Could you check a few things on this model? Use its own coordinates, in mm. Face numbers are marked on the shaded views. A direction names the side the tool comes from. Round coordinates to 2 decimals unless told otherwise and drop trailing zeros. Loops run counter-clockwise (first coordinate to the right, second up) from the corner with the lowest first, then second, coordinate; pieces in that order, holes last. Notation, with made-up numbers: M 13,89 L 54,89 A18 ccw 54,109 Z; hole C 13,19 d5. An arc over 180 degrees is marked long. One line per item, written item: value. Start each with the question number.
Q1. Which directions (+Z, -Z, +X, -X, +Y, -Y) give clear straight access to the entire face, cutting with the end or side of a thin tool? Please do the marked faces 1 and 2.
Q2. Imagine slicing it at A-A (x = 58). Please give me the cut outline in (y, z).
Q3. I'm going to push flat-ended pins straight in: pin 1 Ø2 at (x, y) = (12, 0) entering from -Z; pin 2 Ø2 at (x, z) = (36.5, -3.5) entering from -Y; pin 3 Ø1 at (y, z) = (5, 3.5) entering from -X; pin 4 Ø8 at (x, y) = (38.5, -3) entering from +Z. Where does each tip first touch, or does it pass through?
Q4. Please list where these lines run through material, in increasing order: line 1 along Y through (x, z) = (17.5, -0.25); line 2 along X through (y, z) = (8, 3.5); line 3 along Z through (x, y) = (38.5, -4.5).
from build123d import *

# Parameters (mm, degrees)
BOSS_EXTRUDE_DEPTH = 7.5
CHAMFER_2_SIZE     = 1.4


with BuildPart() as part:
    # Sketch1 → Boss-Extrude (new body)
    with BuildSketch(Plane(origin=(0, 0, 0), x_dir=(0, 0, -1), z_dir=(1, 0, 0))):
        Polygon((9, 5.196152423), (9, -5.196152423), (0, -10.392304845), (-9, -5.196152423), (-9, 5.196152423), (0, 10.392304845), align=None)
    extrude(amount=BOSS_EXTRUDE_DEPTH)

    # Sketch2 → Boss-Revolve1 (revolve)
    with BuildSketch(Plane.XY, mode=Mode.PRIVATE) as boss_revolve1_sk:
        Polygon((0, 0), (62.5, 0), (62.5, 4.4845), (62.5, 6), (7.5, 6), (0, 6), align=None)
    revolve(boss_revolve1_sk.sketch.rotate(Axis((0, 0, 0), (-1, 0, 0)), 90), axis=Axis((0, 0, 0), (-1, 0, 0)))

    # Sketch3 → Cut-Revolve1 (revolve, cut)
    with BuildSketch(Plane.XY):
        Polygon((0, 9), (3.690598923, 15.392304845), (3.690598923, 20.392304845), (-10, 20.392304845), (-10, 9), align=None)
    revolve(axis=Axis((0, 0, 0), (1, 0, 0)), mode=Mode.SUBTRACT)

    # Sketch5 → Cut-Revolve2 (revolve, cut)
    with BuildSketch(Plane.XY):
        Polygon((7.5, 9), (3.809401077, 15.392304845), (3.809401077, 20.392304845), (13.809401077, 20.392304845), (13.809401077, 9), align=None)
    revolve(axis=Axis((0, 0, 0), (1, 0, 0)), mode=Mode.SUBTRACT)

    # Sketch4 → Cut-Revolve3 (revolve, cut)
    with BuildSketch(Plane.XY, mode=Mode.PRIVATE) as cut_revolve3_sk:
        Polygon((7.5, 8.177264973), (6.9, 8.523675135), (6.9, 20.392304845), (7.5, 20.392304845), align=None)
    revolve(cut_revolve3_sk.sketch.rotate(Axis((0, 0, 0), (1, 0, 0)), 90), axis=Axis((0, 0, 0), (1, 0, 0)), mode=Mode.SUBTRACT)

    # Chamfer 2
    chamfer_2_edges = [part.edges().sort_by_distance(p)[0] for p in [
        (62.5, 0, 6),
    ]]
    chamfer(chamfer_2_edges, length=CHAMFER_2_SIZE)

    # Sketch9 → Revolve1 (revolve)
    with BuildSketch(Plane.XY, mode=Mode.PRIVATE) as revolve1_sk:
        with BuildLine():
            Line((7.5, 6.6), (7.5, 6))
            Line((7.5, 6), (8.1, 6))
            ThreePointArc((8.1, 6), (7.675735931, 6.175735931), (7.5, 6.6))
        make_face()
    revolve(revolve1_sk.sketch.rotate(Axis((0, 0, 0), (1, 0, 0)), 90), axis=Axis((0, 0, 0), (1, 0, 0)))


solid = part.part
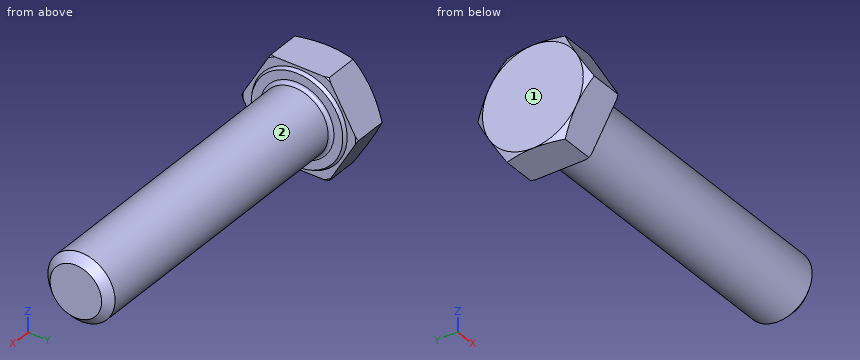
Report:
1. face 1: +Z, -Z, -X, +Y, -Y
1. face 2: +X
2. outline: C 0,0 d12
3. pin 1: stops at z = -6
3. pin 2: stops at y = -5.45
3. pin 3: stops at x = 0
3. pin 4: stops at z = 6
4. line 1: y = -5.99 to 5.99
4. line 2: x = 0 to 6.9
4. line 3: z = -3.97 to 3.97
